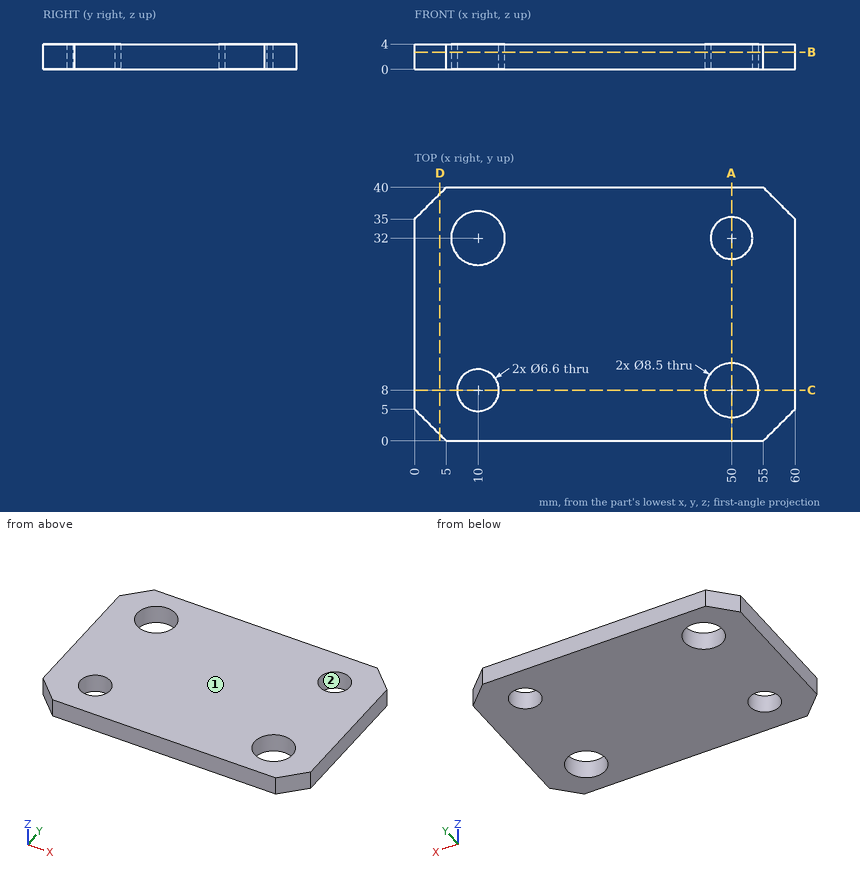
Could you check a few things on this drawing? It's one solid part, dimensions in mm from its lowest x, y, z. Round coordinates to 2 decimals unless told otherwise and drop trailing zeros. Loops run counter-clockwise (first coordinate to the right, second up) from the corner with the lowest first, then second, coordinate; pieces in that order, holes last. Notation, with made-up numbers: M 1,-6 L 13,-6 A21 ccw 13,23 Z; hole C 45,-12 d8. An arc over 180 degrees is marked long. Write each question's results on one line, items separated by ' | '. Start each with the question number.
(1) I want a section at B-B (z = 2.7). Please give me the cut outline in (x, y).
(2) If I drill on probe 1 along Y at (x, z) = (50, 2.3); probe 2 along Y at (x, z) = (10, 1.1); probe 3 along X at (y, z) = (9, 1.8), over which ranges is the centre line in solid material (lowest first)? Write a range as from..to.
(3) I want a section at C-C (y = 8). Please give me the cut outline in (x, z).
(4) Will this pin go through, and if not, where does the flat tip stop? P1, Ø11, axis at x = 10, y = 32, coming from the +Z side.
(5) I want a section at D-D (x = 4). Please give me the cut outline in (y, z), then the cut area to 3 significant figures.
(6) Thinking about a two-plate mould opening in Y: for the marked faces 1 and 2, which applies, pulls with the +Y half, pulls with the -Y half, needs draft (parallel to the pull), parting line crosses it, or undercut?
(7) I want a section at A-A (x = 50). Please give me the cut outline in (y, z), then the cut area to 3 significant figures.
Solved:
1) outline: M 0,5 L 5,0 L 55,0 L 60,5 L 60,35 L 55,40 L 5,40 L 0,35 Z; hole C 10,32 d8.5; hole C 10,8 d6.6; hole C 50,8 d8.5; hole C 50,32 d6.6
2) probe 1: y = 0..3.75, 12.25..28.7, 35.3..40 | probe 2: y = 0..4.7, 11.3..27.75, 36.25..40 | probe 3: x = 0..6.86, 13.14..45.87, 54.13..60
3) outline: M 0,0 L 6.7,0 L 6.7,4 L 0,4 Z; M 13.3,0 L 45.75,0 L 45.75,4 L 13.3,4 Z; M 54.25,0 L 60,0 L 60,4 L 54.25,4 Z
4) P1: stops at z = 4
5) outline: M 1,0 L 39,0 L 39,4 L 1,4 Z | area: 152 mm²
6) face 1: needs draft | face 2: undercut
7) outline: M 0,0 L 3.75,0 L 3.75,4 L 0,4 Z; M 12.25,0 L 28.7,0 L 28.7,4 L 12.25,4 Z; M 35.3,0 L 40,0 L 40,4 L 35.3,4 Z | area: 99.6 mm²
